from build123d import *

# Parameters (mm, degrees)
L_SIDE_WALL_DEPTH            = 15
BASE_FLANGE_WITH_TAB_DEPTH   = 15
UPRIGHT_PLATE_SKETCH_W       = 75
UPRIGHT_PLATE_SKETCH_H       = 15
UPRIGHT_PLATE_DEPTH          = 60
UPRIGHT_CROSS_HOLE_SKETCH_R  = 10
UPRIGHT_CROSS_HOLE_DEPTH     = 118.68177429
TAB_MOUNTING_HOLE_DEPTH      = 111.788086002
TAB_MOUNTING_HOLE_DEPTH_BACK = 111.788086002
TAB_MOUNTING_HOLE_SKETCH_R   = 6.5


with BuildPart() as part:
    # L Side Wall Sketch → L Side Wall (new body)
    with BuildSketch(Plane.XY):
        Polygon((0, 0), (0, 60), (-75, 60), (-75, 45), (-25, 45), (-25, 0), align=None)
    extrude(amount=-L_SIDE_WALL_DEPTH)

    # Base Flange Sketch → Base Flange With Tab (add)
    with BuildSketch(Plane(origin=(0, 0, 0), x_dir=(1, 0, 0), z_dir=(0, 1, 0))):
        Polygon((25, 68), (25, 38), (0, 38), (0, 0), (-25, 0), (-25, 53), (0, 53), (0, 68), align=None)
    extrude(amount=BASE_FLANGE_WITH_TAB_DEPTH)

    # Upright Plate Sketch → Upright Plate (add)
    with BuildSketch(Plane(origin=(0, 0, 0), x_dir=(1, 0, 0), z_dir=(0, 1, 0))):
        with Locations((-37.5, 60.5)):
            Rectangle(UPRIGHT_PLATE_SKETCH_W, UPRIGHT_PLATE_SKETCH_H)
    extrude(amount=UPRIGHT_PLATE_DEPTH)

    # Upright Cross Hole Sketch → Upright Cross Hole (cut, through all)
    with BuildSketch(Plane(origin=(0, 0, -68), x_dir=(-1, 0, 0), z_dir=(0, 0, -1))):
        with Locations((45, 30)):
            Circle(UPRIGHT_CROSS_HOLE_SKETCH_R)
    extrude(amount=-UPRIGHT_CROSS_HOLE_DEPTH, mode=Mode.SUBTRACT)

    # Tab Mounting Hole Sketch → Tab Mounting Hole (cut, two sides: drawn at the far end of the back side and taken through both)
    with BuildSketch(Plane(origin=(0, 15, 0), x_dir=(1, 0, 0), z_dir=(0, 1, 0)).offset(-TAB_MOUNTING_HOLE_DEPTH_BACK)):
        with Locations(Location((13, 53, 0), (0, 0, 270))):
            Circle(TAB_MOUNTING_HOLE_SKETCH_R)
    extrude(amount=TAB_MOUNTING_HOLE_DEPTH + TAB_MOUNTING_HOLE_DEPTH_BACK, mode=Mode.SUBTRACT)


solid = part.part
Part model, mm, in its own coordinate system. A direction names the side the tool comes from. Coordinates: 2 decimals unless noted, no trailing zeros. Write each loop counter-clockwise with the first axis right and the second up, starting at its lowest first coordinate (ties: lowest second). Pieces come first, ordered by that corner, then holes. Notation, with made-up numbers: M 84,50.5 L 98,50.5 A16 cw 98,74.5 Z; hole C 15.25,-14 d1. An arc over 180 degrees is marked long. Return JSON: item names as keys, results as strings.
1. Flat gauge pins, fed straight in: pin 1 Ø11.5 at (y, z) = (31.5, -18) entering from +X; pin 2 Ø13.5 at (y, z) = (33.5, -27.5) entering from -X; pin 3 Ø12 at (x, z) = (-47.5, -7) entering from -Y; pin 4 Ø15 at (x, z) = (13, -53) entering from +Y. Where does each tip first touch, or does it go through?
Determined:
{"pin 1": "x = 0", "pin 2": "through", "pin 3": "y = 45", "pin 4": "y = 15"}
2. Probe L1, parallel to Y at x = -45.5, z = -54.5; L2, parallel to Z at x = 13, y = 6; L3, parallel to Z at x = -14.5, y = 23. List the from-to ranges inside material, lowest first.
Determined:
{"L1": "0 to 20.01, 39.99 to 60", "L2": "-68 to -59.5, -46.5 to -38", "L3": "-68 to -53, -15 to 0"}
3. Pull direction Z, two halves, no side cores. Call faces 1 (the face through (-37, 23, -68)), 2 (the face through (14.95, 7.39, -46.8)), 3 (the face through (-15, 0, -50)), 4 (the face through (-21, 37, 0)): pulls with the +Z half, pulls with the -Z half, needs draft (parallel to the pull), parting line crosses it, or undercut.
Determined:
{"face 1": "pulls with the -Z half", "face 2": "undercut", "face 3": "needs draft", "face 4": "pulls with the +Z half"}
4. Saw through at A-A, the plane y = 52.5. Write the cut outline in (x, z), then the cut area to 3 significant figures.
Determined:
{"outline": "M -75,-68 L 0,-68 L 0,-53 L -75,-53 Z; M -75,-15 L 0,-15 L 0,0 L -75,0 Z", "area": "2,250 mm²"}
5. Saw through at D-D, the plane x = -45. Write the cut outline in (y, z), then the cut area to 3 significant figures.
Determined:
{"outline": "M 0,-68 L 20,-68 L 20,-53 L 0,-53 Z; M 40,-68 L 60,-68 L 60,-53 L 40,-53 Z; M 45,-15 L 60,-15 L 60,0 L 45,0 Z", "area": "825 mm²"}
6. 3-axis set-ups, long thin cutter, end or side, ignore diameter. For faces 5 (the face through (-30, 48, -15)), 6 (the face through (13, 7, -38)), 7 (the face through (-30, 30, -53)), 8 (the face through (-25, 12, -20)): which of +Z, -Z, +X, -X, +Y, -Y reach the whole face in a straight line?
Determined:
{"face 5": "+X, -X, +Y", "face 6": "+Z, +X, +Y, -Y", "face 7": "-X, +Y", "face 8": "+Z, -X, -Y"}
7. Saw through at C-C, the plane y = 30. Write the cut outline in (x, z), then the cut area to 3 significant figures.
Determined:
{"outline": "M -75,-68 L -55,-68 L -55,-53 L -75,-53 Z; M -35,-68 L 0,-68 L 0,-53 L -35,-53 Z; M -25,-15 L 0,-15 L 0,0 L -25,0 Z", "area": "1,200 mm²"}
8. Saw through at B-B, the plane x = 13. Write the cut outline in (y, z).
Determined:
{"outline": "M 0,-68 L 15,-68 L 15,-59.5 L 0,-59.5 Z; M 0,-46.5 L 15,-46.5 L 15,-38 L 0,-38 Z"}
